Work out the finished part from the listing and answer in its coordinate system (mm). A direction names the side the tool comes from. Coordinates: 2 decimals unless noted, no trailing zeros. Write each loop counter-clockwise with the first axis right and the second up, starting at its lowest first coordinate (ties: lowest second). Pieces come first, ordered by that corner, then holes. Notation, with made-up numbers: (75.25, 19) - (100.25, 19) arc R13 cw to (100.25, 25) - close; hole circle Ø3 at (75, 62). An arc over 180 degrees is marked (long way). Use a Markdown table: item, result. Add a question column.
(1) The part is cut by section C-C, the plane z = -7.5. Give the vertices of the cut face in (x, y), then the cut area to 3 significant figures.
(2) A tool of negligible diameter and unlimited length cuts with its end or side. For faces 1 (the face through (0, 15, 1)), 2 (the face through (0, 12, 1)), from which of +Z, -Z, +X, -X, +Y, -Y can it reach the whole face along a straight path? Write none if from no direction.
(3) Find the intervals of material crossed by line 1 (X direction, y = -5, z = 8.5); line 2 (Y direction, x = -11.5, z = 63), in increasing order. Write a range as from..to.
(4) For a pull along Y with two mould halves and no side action, classify faces 3 (the face through (13.797, 13.859, 1.19)), 4 (the face through (14, 0, -85)), 5 (the face through (-12, 0, 1)), 6 (the face through (12, 0, 1)) as released by +Y, released by -Y, zero draft, split by the parting line, or undercut.
(5) The part is cut by section A-A, the plane y = 3.5. Give the vertices of the cut face in (x, z), then the cut area to 3 significant figures.
from build123d import *

# Parameters (mm, degrees)
EXTRUDE_1_DEPTH = 85


with BuildPart() as part:
    # 草图2 → 拉伸-薄壁1 (new, symmetric)
    with BuildSketch(Plane.XY):
        with BuildLine():
            Line((-11, 15), (11, 15))
            ThreePointArc((11, 15), (13.828427125, 13.828427125), (15, 11))
            Line((15, 11), (15, -11))
            ThreePointArc((15, -11), (13.828427125, -13.828427125), (11, -15))
            Line((11, -15), (-11, -15))
            ThreePointArc((-11, -15), (-13.828427125, -13.828427125), (-15, -11))
            Line((-15, -11), (-15, 11))
            ThreePointArc((-15, 11), (-13.828427125, 13.828427125), (-11, 15))
        make_face()
        with BuildLine():
            Line((-11, 12), (11, 12))
            ThreePointArc((11, 12), (11.707106781, 11.707106781), (12, 11))
            Line((12, 11), (12, -11))
            ThreePointArc((12, -11), (11.707106781, -11.707106781), (11, -12))
            Line((11, -12), (-11, -12))
            ThreePointArc((-11, -12), (-11.707106781, -11.707106781), (-12, -11))
            Line((-12, -11), (-12, 11))
            ThreePointArc((-12, 11), (-11.707106781, 11.707106781), (-11, 12))
        make_face(mode=Mode.SUBTRACT)
    extrude(amount=EXTRUDE_1_DEPTH, both=True)


solid = part.part
Model answer:
| question | item | result |
|---|---|---|
| 1 | outline | (-15, -11) arc R4 ccw to (-11, -15) - (11, -15) arc R4 ccw to (15, -11) - (15, 11) arc R4 ccw to (11, 15) - (-11, 15) arc R4 ccw to (-15, 11) - close; hole (-12, -11) arc R1 ccw to (-11, -12) - (11, -12) arc R1 ccw to (12, -11) - (12, 11) arc R1 ccw to (11, 12) - (-11, 12) arc R1 ccw to (-12, 11) - close |
| 1 | area | 311 mm^2 |
| 2 | face 1 | +Z, -Z, +X, -X, +Y |
| 2 | face 2 | +Z, -Z |
| 3 | line 1 | -15..-12, 12..15 |
| 3 | line 2 | -14.97..-11.87, 11.87..14.97 |
| 4 | face 3 | released by +Y |
| 4 | face 4 | zero draft |
| 4 | face 5 | undercut |
| 4 | face 6 | undercut |
| 5 | outline | (-15, -85) - (-12, -85) - (-12, 85) - (-15, 85) - close; (12, -85) - (15, -85) - (15, 85) - (12, 85) - close |
| 5 | area | 1,020 mm^2 |
